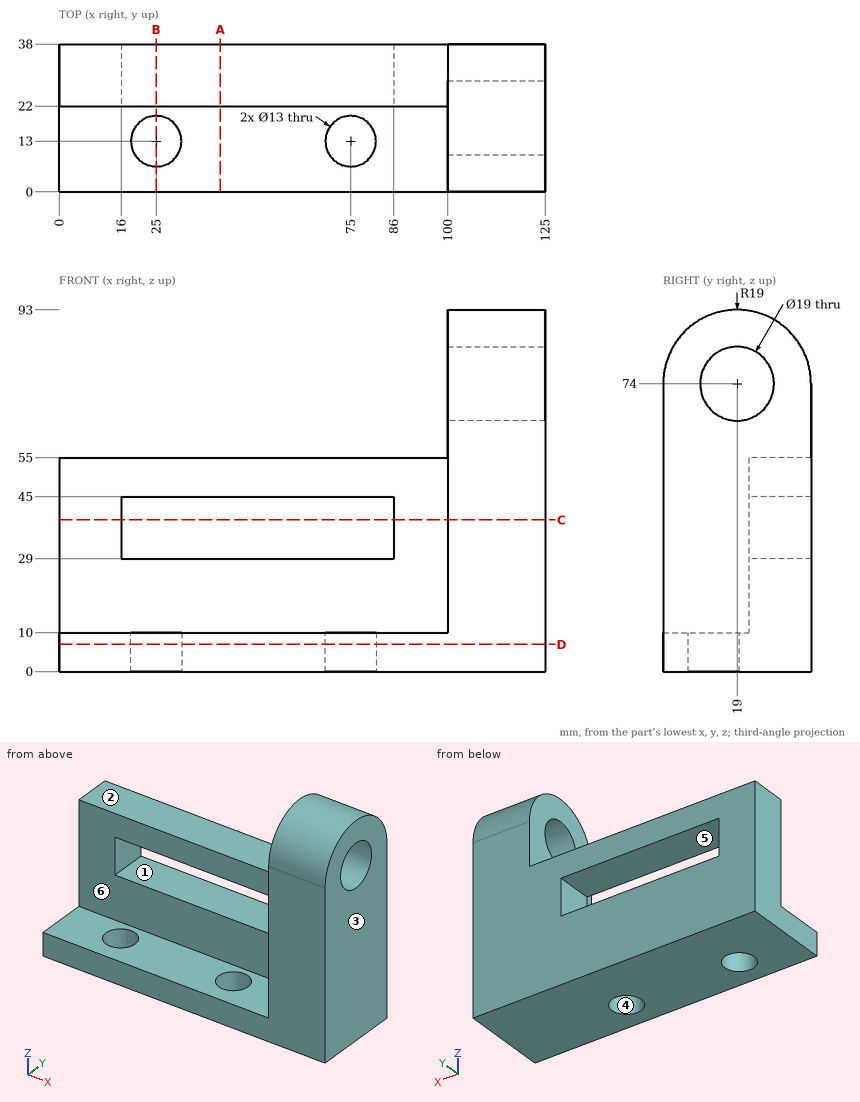
Could you check a few things on this drawing? It's one solid part, dimensions in mm from its lowest x, y, z. A direction names the side the tool comes from. Give positions to 0.01 mm unless a question says otherwise; leave off trailing zeros. Order: outer loops, then holes, each group sorted by start corner. A loop starts at its lowest first (then second) coordinate and runs counter-clockwise, first axis right, second up.
1. Suppose I cut it at B-B (x = 25). Write out the boundary of the cut face in (y, z).
Answers below:
outline: (0, 0) - (6.5, 0) - (6.5, 10) - (0, 10) - close; (19.5, 0) - (38, 0) - (38, 29) - (22, 29) - (22, 10) - (19.5, 10) - close; (22, 45) - (38, 45) - (38, 55) - (22, 55) - close
2. Thinking about a two-plate mould opening in X: for the marked faces 1, 2 and 3, which applies, +X half, -X half, draft (parallel to the pull), parting line (faces both ways), or undercut?
Answers below:
face 1: undercut
face 2: draft
face 3: +X half
3. I need wall thicknesses on L1, parallel to Y at x = 119.5, z = 74; L2, parallel to Z at x = 57, y = 24; L3, parallel to X at y = 32, z = 30.5. Which ranges of each line are inside material? Lowest first, please.
Answers below:
L1: y = 0 to 9.5, 28.5 to 38
L2: z = 0 to 29, 45 to 55
L3: x = 0 to 16, 86 to 125
4. Suppose I cut it at A-A (x = 41.5). Write out the boundary of the cut face in (y, z), plus the area to 3 significant figures.
Answers below:
outline: (0, 0) - (38, 0) - (38, 29) - (22, 29) - (22, 10) - (0, 10) - close; (22, 45) - (38, 45) - (38, 55) - (22, 55) - close
area: 844 mm2
5. Which directions (+Z, -Z, +X, -X, +Y, -Y) give clear straight access to the entire face, cutting with the end or side of a thin tool? Please do the marked faces 4, 5 and 6.
Answers below:
face 4: +Z, -Z
face 5: +Y, -Y
face 6: +Z, -X, -Y
6. Suppose I cut it at C-C (z = 39). Write out the boundary of the cut face in (x, y).
Answers below:
outline: (0, 22) - (16, 22) - (16, 38) - (0, 38) - close; (86, 22) - (100, 22) - (100, 0) - (125, 0) - (125, 38) - (86, 38) - close
7. For pin 1 (11.5 mm diameter, centred on y = 16.5, z = 63.5, fed in from -X); pin 2 (8 mm diameter, centred on x = 63, y = 29, fed in from +Z); pin 3 (17 mm diameter, centred on x = 75, y = 13, fed in from +Z), each with a flat end and sliding along its axis, tell me the tip position at first contact or that it passes through.
Answers below:
pin 1: stops at x = 100
pin 2: stops at z = 55
pin 3: stops at z = 10
8. Suppose I cut it at D-D (z = 7). Write out the boundary of the cut face in (x, y).
Answers below:
outline: (0, 0) - (125, 0) - (125, 38) - (0, 38) - close; hole circle Ø13 at (25, 13); hole circle Ø13 at (75, 13)
